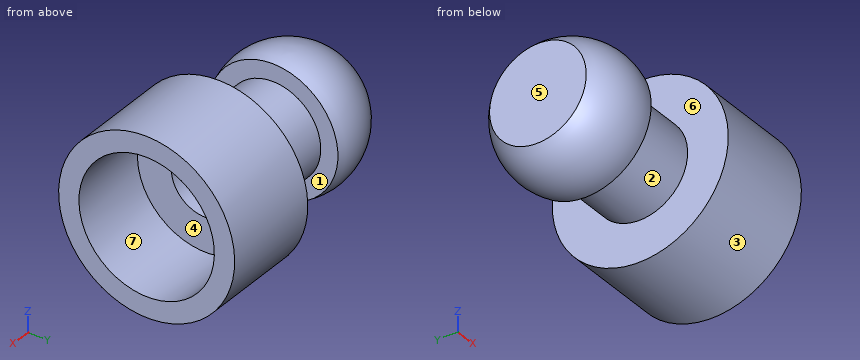
from build123d import *


with BuildPart() as part:
    # Sketch1 → Revolve1 (revolve)
    with BuildSketch(Plane(origin=(0, 0, 0), x_dir=(-1, 0, 0), z_dir=(0, 0, -1)), mode=Mode.PRIVATE) as revolve1_sk:
        with BuildLine():
            Line((21, 5), (23.886751346, 0))
            Line((23.886751346, 0), (36, 0))
            Line((36, 0), (36, 7.141428429))
            ThreePointArc((36, 7.141428429), (31.331857058, 9.724322221), (26, 9.539392014))
            Line((26, 9.539392014), (26, 7))
            Line((26, 7), (15, 7))
            Line((15, 7), (15, 13))
            Line((15, 13), (0, 13))
            Line((0, 13), (0, 10))
            Line((0, 10), (12, 10))
            Line((12, 10), (12, 5))
            Line((12, 5), (21, 5))
        make_face()
    revolve(revolve1_sk.sketch.rotate(Axis((0, 0, 0), (-1, 0, 0)), 270), axis=Axis((0, 0, 0), (-1, 0, 0)))


solid = part.part
Can you work these out from the model? Positions are in its coordinate system, mm. Face numbers are marked on the shaded views. A direction names the side the tool comes from. Coordinates: 2 decimals unless noted, no trailing zeros. Loops run counter-clockwise (first coordinate to the right, second up) from the corner with the lowest first, then second, coordinate; pieces in that order, holes last. Notation, with made-up numbers: (-27.75, 72.25) - (6.25, 72.25) arc R13 cw to (6.25, 87.25) - close; hole circle Ø5 at (-35.75, 28). An arc over 180 degrees is marked (long way). Answer as a JSON object with one key per item and string values. Group by question number.
Item 1: If I drill on L1, parallel to Y at x = -17, z = 0; L2, parallel to Y at x = -7.25, z = 0; L3, parallel to X at y = 5.5, z = -4.75, over which ranges is the centre line in solid material (lowest first)? Write a range as from..to.
Item 2: For pin 1 (6 mm diameter, centred on x = -22.5, y = 5, fed in from +Z); pin 2 (1.5 mm diameter, centred on x = -25, y = -2.5, fed in from -Z); pin 3 (6 mm diameter, centred on y = 2, z = -4, fed in from +X), each with a flat end and sliding along its axis, tell me the tip position at first contact or that it passes through.
Item 3: On a 3-axis mill with a long thin cutter (end or side, diameter ignored), from which of +Z, -Z, +X, -X, +Y, -Y can I reach the whole of each face in a straight line? I mean the marked faces 5, 6 and 7. Say none if no direction works.
Item 4: If we section it at B-B (y = 9): List the corners of the cut face in (x, z) for me.
Item 5: If we section it at C-C (x = -18): List the corners of the cut face in (y, z) for me.
Item 6: If we section it at A-A (z = -8): List the corners of the cut face in (x, y) for me, plus the area to 3 significant figures.
Item 7: If we section it at D-D (y = -10.5): List the corners of the cut face in (x, z) for me.
Item 8: If we mould it in two halves opening along X, with no side actions, what happens to the marked faces 1, 2, 3 and 4? For each: released by +X, released by -X, zero draft, split by the parting line, or undercut.
Returned:
{
 "1": {"L1": "y = -7..-5, 5..7", "L2": "y = -13..-10, 10..13", "L3": "x = -35.87..-26, -15..-12"},
 "2": {"pin 1": "stops at z = 6.71", "pin 2": "stops at z = -6.78", "pin 3": "stops at x = -12"},
 "3": {"face 5": "+Z, -Z, -X, +Y, -Y", "face 6": "none", "face 7": "+X"},
 "4": {"outline": "(-26, -3.16) - (-26, 3.16) arc R4.36 ccw (long way) to start; (-15, -9.38) - (0, -9.38) - (0, -4.36) - (-12, -4.36) - (-12, 4.36) - (0, 4.36) - (0, 9.38) - (-15, 9.38) - close"},
 "5": {"outline": "circle Ø14 at (0, 0); hole circle Ø10 at (0, 0)"},
 "6": {"outline": "(-26, -5.2) - (-26, 5.2) arc R6 ccw (long way) to start; (-15, -10.25) - (0, -10.25) - (0, -6) - (-12, -6) - (-12, 6) - (0, 6) - (0, 10.25) - (-15, 10.25) - close", "area": "254 mm²"},
 "7": {"outline": "(-15, -7.66) - (0, -7.66) - (0, 7.66) - (-15, 7.66) - close"},
 "8": {"face 1": "undercut", "face 2": "undercut", "face 3": "zero draft", "face 4": "released by +X"}
}
